Could you check a few things on this model? Use its own coordinates, in mm. Face numbers are marked on the shaded views. A direction names the side the tool comes from. Give positions to 0.01 mm unless a question says otherwise; leave off trailing zeros. Loops run counter-clockwise (first coordinate to the right, second up) from the corner with the lowest first, then second, coordinate; pieces in that order, holes last. Notation, with made-up numbers: (31.5, 1.25) -> (48.5, 1.25) arc R21 ccw to (48.5, 40.25) -> close; hole circle Ø5 at (-15, -19.75). An arc over 180 degrees is marked (long way). Write item = value, one per line. Start each with the question number.
1) I need wall thicknesses on probe 1 along X at (y, z) = (35.5, 7); probe 2 along Z at (x, y) = (-67.5, 33); probe 3 along Y at (x, z) = (-48, -19.5). Which ranges of each line are inside material? Lowest first, please. Write a range as from..to.
2) If we mould it in two halves opening along Z, with no side actions, what happens to the marked faces 1, 2, 3 and 4? For each: +Z half, -Z half, draft (parallel to the pull), parting line (faces both ways), or undercut.
3) I want a section at D-D (z = 11.5). List the corners of the cut face in (x, y) for me.
4) I want a section at A-A (y = -80). List the corners of the cut face in (x, z) for me, and give its area (3 significant figures).
5) I'm going to push flat-ended pins straight in: pin 1 Ø8 at (x, z) = (-8.5, 0) entering from +Y; pin 2 Ø4 at (x, z) = (-51.5, 10.5) entering from -Y; pin 3 Ø5 at (x, y) = (-16, -18.5) entering from -Z. Where does each tip first touch, or does it pass through?
6) I want a section at B-B (x = -53.5). List the corners of the cut face in (y, z) for me, and give its area (3 significant figures).
7) I want a section at C-C (z = -11.5). List the corners of the cut face in (x, y) for me, and give its area (3 significant figures).
8) On a 3-axis mill with a long thin cutter (end or side, diameter ignored), from which of +Z, -Z, +X, -X, +Y, -Y can I reach the whole of each face in a straight line? I mean the marked faces 5, 6 and 7. Say none if no direction works.
from build123d import *
from build123d.topology import SkipClean

# Parameters (mm, degrees)
BRACKET_PROFILE_SKETCH_R       = 10.5
BRACKET_BODY_145MM_DEPTH       = 72.5
PLATE_AND_LUG_OUTLINE_SKETCH_R = 7.5
PLATE_AND_LUG_OUTLINE_SKETCH_W = 101
PLATE_AND_LUG_OUTLINE_SKETCH_H = 63.401381975
OUTLINE_AND_HOLES_CUT_DEPTH    = 145
LUG_REGION_BOSS_DEPTH          = 20


with BuildPart() as part:
    # Bracket Profile Sketch → Bracket Body 145mm (new, symmetric)
    with BuildSketch(Plane(origin=(0, 0, 0), x_dir=(0, 0, -1), z_dir=(1, 0, 0))):
        with BuildLine():
            Line((-8.607818135, 33), (-8.607818135, -0.114515686))
            Line((-8.607818135, -0.114515686), (-20, -0.114515686))
            Line((-20, -0.114515686), (-20, -75.114515686))
            Line((-20, -75.114515686), (0, -75.114515686))
            Line((0, -75.114515686), (0, 0))
            Line((0, 0), (33.392181865, 0))
            Line((33.392181865, 0), (33.392181865, 33))
            ThreePointArc((33.392181865, 33), (12.392181865, 54), (-8.607818135, 33))
        make_face()
        with Locations((12.392181865, 33)):
            Circle(BRACKET_PROFILE_SKETCH_R, mode=Mode.SUBTRACT)
    extrude(amount=BRACKET_BODY_145MM_DEPTH, both=True)

    # Plate and Lug Outline Sketch → Outline and Holes Cut (cut)
    with BuildSketch(Plane.XY.offset(20)):
        with BuildLine():
            Line((-38.846882472, -75.114515686), (-62.792895003, -61.686845107))
            ThreePointArc((-62.792895003, -61.686845107), (-69.894587599, -54.717509879), (-72.5, -45.114515686))
            Line((-72.5, -45.114515686), (-72.5, -75.114515686))
            Line((-72.5, -75.114515686), (-38.846882472, -75.114515686))
        make_face()
        with BuildLine():
            Line((62.792895003, -61.686845107), (38.846882472, -75.114515686))
            Line((38.846882472, -75.114515686), (72.5, -75.114515686))
            Line((72.5, -75.114515686), (72.5, -45.114515686))
            ThreePointArc((72.5, -45.114515686), (69.894587599, -54.717509879), (62.792895003, -61.686845107))
        make_face()
        with Locations((53.5, -45.114515686)):
            Circle(PLATE_AND_LUG_OUTLINE_SKETCH_R)
        with BuildLine():
            ThreePointArc((0, -67.614515686), (-5.303300859, -69.811214827), (-7.5, -75.114515686))
            Line((-7.5, -75.114515686), (0, -75.114515686))
            Line((0, -75.114515686), (0, -67.614515686))
        make_face()
        with BuildLine():
            ThreePointArc((7.5, -75.114515686), (5.303300859, -69.811214827), (0, -67.614515686))
            Line((0, -67.614515686), (0, -75.114515686))
            Line((0, -75.114515686), (7.5, -75.114515686))
        make_face()
        with BuildLine():
            Line((0, -75.114515686), (-7.5, -75.114515686))
            ThreePointArc((-7.5, -75.114515686), (0, -82.614515686), (7.5, -75.114515686))
            Line((7.5, -75.114515686), (0, -75.114515686))
        make_face()
        with Locations((-53.5, -45.114515686)):
            Circle(PLATE_AND_LUG_OUTLINE_SKETCH_R)
        with Locations((0, 43.586175301)):
            Rectangle(PLATE_AND_LUG_OUTLINE_SKETCH_W, PLATE_AND_LUG_OUTLINE_SKETCH_H)
    extrude(amount=-OUTLINE_AND_HOLES_CUT_DEPTH, mode=Mode.SUBTRACT)

    # Sketch2_3 → Lug Region Boss (add)
    with SkipClean():  # the faces are left unmerged after this step: merging them gives an invalid solid
        with BuildSketch(Plane.XY.offset(20)):
            with BuildLine():
                Line((-7.5, -75.114515686), (-38.846882472, -75.114515686))
                Line((-38.846882472, -75.114515686), (-9.292895003, -91.686845107))
                ThreePointArc((-9.292895003, -91.686845107), (0, -94.114515686), (9.292895003, -91.686845107))
                Line((9.292895003, -91.686845107), (38.846882472, -75.114515686))
                Line((38.846882472, -75.114515686), (7.5, -75.114515686))
                ThreePointArc((7.5, -75.114515686), (0, -82.614515686), (-7.5, -75.114515686))
            make_face()
        extrude(amount=-LUG_REGION_BOSS_DEPTH)


solid = part.part
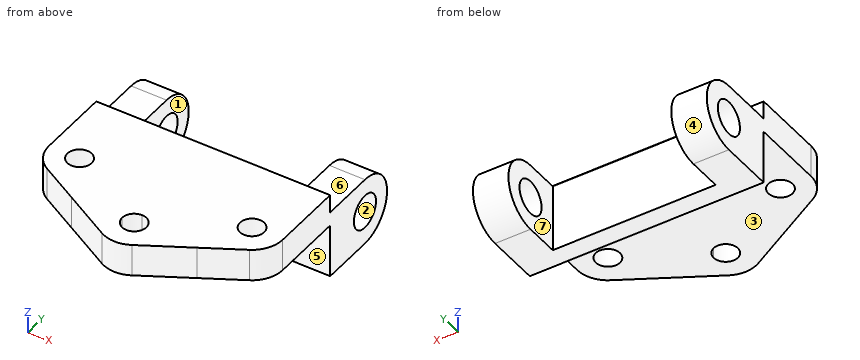
Answer list:
q1.probe_1 = -72.5..-50.5, 50.5..72.5
q1.probe_2 = -33.39..-22.89, -1.89..8.61
q1.probe_3 = 0..11.89
q2.face_1 = draft
q2.face_2 = undercut
q2.face_3 = -Z half
q2.face_4 = parting line
q3.outline = (-72.5, -45.11) arc R19 ccw to (-62.79, -61.69) -> (-9.29, -91.69) arc R19 ccw to (9.29, -91.69) -> (62.79, -61.69) arc R19 ccw to (72.5, -45.11) -> (72.5, -0.11) -> (-72.5, -0.11) -> close; hole circle Ø15 at (-53.5, -45.11); hole circle Ø15 at (0, -75.11); hole circle Ø15 at (53.5, -45.11)
q4.outline = (-30.13, 0) -> (-5.69, 0) -> (-5.69, 20) -> (-30.13, 20) -> close; (5.69, 0) -> (30.13, 0) -> (30.13, 20) -> (5.69, 20) -> close
q4.area = 978 mm^2
q5.pin_1 = 11.89
q5.pin_2 = -69.14
q5.pin_3 = 0
q6.outline = (-66.9, 0) -> (-52.61, 0) -> (-52.61, 20) -> (-66.9, 20) -> close; (-37.61, 0) -> (0, 0) -> (0, -33.39) -> (33, -33.39) arc R21 ccw to (33, 8.61) -> (-0.11, 8.61) -> (-0.11, 20) -> (-37.61, 20) -> close; hole circle Ø21 at (33, -12.39)
q6.area = 2,770 mm^2
q7.outline = (-72.5, 0) -> (72.5, 0) -> (72.5, 22.54) -> (50.5, 22.54) -> (50.5, 11.89) -> (-50.5, 11.89) -> (-50.5, 22.54) -> (-72.5, 22.54) -> close; (-72.5, 43.46) -> (-50.5, 43.46) -> (-50.5, 53.98) -> (-72.5, 53.98) -> close; (50.5, 43.46) -> (72.5, 43.46) -> (72.5, 53.98) -> (50.5, 53.98) -> close
q7.area = 2,650 mm^2
q8.face_5 = -Z, +X, -X, -Y
q8.face_6 = +Z, +X, -X, +Y
q8.face_7 = +Z, -Z, +Y
